from build123d import *

# Parameters (mm, degrees)
SKETCH1_R           = 60
SKETCH1_R_2         = 55
BOSS_EXTRUDE1_DEPTH = 20
CUT_EXTRUDE1_START  = -10
SKETCH2_R           = 60
SKETCH2_R_2         = 58
CUT_EXTRUDE1_DEPTH  = 10
SKETCH3_R           = 60
SKETCH3_R_2         = 55
BOSS_EXTRUDE2_DEPTH = 10
CHAMFER1_SIZE       = 2
CHAMFER2_SIZE       = 1


with BuildPart() as part:
    # Sketch1 → Boss-Extrude1 (new body)
    with BuildSketch(Plane.XY):
        Circle(SKETCH1_R)
        Circle(SKETCH1_R_2, mode=Mode.SUBTRACT)
    extrude(amount=BOSS_EXTRUDE1_DEPTH)

    # Sketch2 → Cut-Extrude1 (cut)
    with BuildSketch(Plane.XY.offset(20).offset(CUT_EXTRUDE1_START)):
        Circle(SKETCH2_R)
        Circle(SKETCH2_R_2, mode=Mode.SUBTRACT)
    extrude(amount=CUT_EXTRUDE1_DEPTH, mode=Mode.SUBTRACT)

    # Sketch3 → Boss-Extrude2 (add)
    with BuildSketch(Plane.XY.offset(20)):
        Circle(SKETCH3_R)
        Circle(SKETCH3_R_2, mode=Mode.SUBTRACT)
    extrude(amount=BOSS_EXTRUDE2_DEPTH)

    # Chamfer1
    chamfer1_edges = [part.edges().sort_by_distance(p)[0] for p in [
        (-60, 0, 0),
    ]]
    chamfer(chamfer1_edges, length=CHAMFER1_SIZE)

    # Chamfer2
    chamfer2_edges = [part.edges().sort_by_distance(p)[0] for p in [
        (-60, 0, 10),
    ]]
    chamfer(chamfer2_edges, length=CHAMFER2_SIZE)


solid = part.part
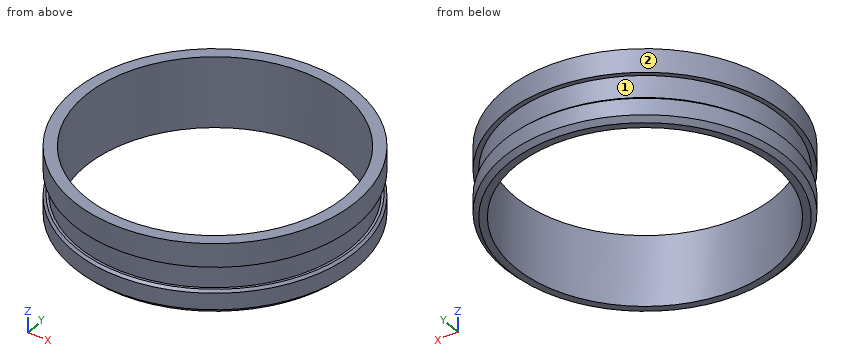
The model under review builds one solid part; all positions refer to its coordinate system, in mm. Face numbers are marked on the shaded views. Give positions to 0.01 mm unless a question says otherwise; leave off trailing zeros. Write each loop counter-clockwise with the first axis right and the second up, starting at its lowest first coordinate (ties: lowest second). Pieces come first, ordered by that corner, then holes.
1. Wall thickness on L1, parallel to Y at x = 0, z = 21.25; L2, parallel to Y at x = 0, z = 16; L3, parallel to X at y = 6.5, z = 25.75: over which ranges is each line inside the solid? List them lowest first.
2. Add section C-C, the plane z = 27. Write out the cut boundary in (x, y), plus the area to 3 significant figures.
3. Draft analysis for pull direction Z (two halves, no side actions). For the marked faces 1 and 2, state which applies: +Z half, -Z half, draft (parallel to the pull), parting line (faces both ways), or undercut.
4. Add section A-A, the plane x = 0. Write out the cut boundary in (y, z), plus the area to 3 significant figures.
5. For P1, Ø5, axis at y = -29, z = 20.5, coming from the +X side; P2, Ø6, axis at x = -3, z = 6, coming from the +Y side; P3, Ø1, axis at y = -12.5, z = 25, coming from the -X side, all flat-tipped, find the tip position at first contact; note any pin that passes through.
Worked answers:
1. L1: y = -60 to -55, 55 to 60
1. L2: y = -58 to -55, 55 to 58
1. L3: x = -59.65 to -54.61, 54.61 to 59.65
2. outline: circle Ø120 at (0, 0); hole circle Ø110 at (0, 0)
2. area: 1,810 mm2
3. face 1: undercut
3. face 2: draft
4. outline: (-60, 2) - (-58, 0) - (-55, 0) - (-55, 30) - (-60, 30) - (-60, 20) - (-58, 20) - (-58, 10) - (-59, 10) - (-60, 9) - close; (55, 0) - (58, 0) - (60, 2) - (60, 9) - (59, 10) - (58, 10) - (58, 20) - (60, 20) - (60, 30) - (55, 30) - close
4. area: 255 mm2
5. P1: stops at x = 53.83
5. P2: stops at y = 60
5. P3: stops at x = -58.79
